```python
from build123d import *
from OCP.BRepFilletAPI import BRepFilletAPI_MakeChamfer

# Parameters (mm, degrees)
SKETCH1_R        = 10.376
BASENUT_DEPTH    = 38
ENDCHAMFER_SIZE  = 1.0376
ENDCHAMFER_SIZE2 = 0.599058639


with BuildPart() as part:
    # Sketch1 → BaseNut (new body)
    with BuildSketch(Plane.XY):
        Polygon((10.392304845, -18), (20.784609691, 0), (10.392304845, 18), (-10.392304845, 18), (-20.784609691, 0), (-10.392304845, -18), align=None)
        Circle(SKETCH1_R, mode=Mode.SUBTRACT)
    extrude(amount=-BASENUT_DEPTH)

    # Sketch2 → Double-Chamfer (revolve, cut)
    with BuildSketch(Plane(origin=(0, 0, 0), x_dir=(1, 0, 0), z_dir=(0, 1, 0))):
        Polygon((-20.784609691, 38), (-17.625, 38), (-20.784609691, 36.175798494), align=None)
        Polygon((-20.784609691, 1.824201506), (-20.784609691, 0), (-17.625, 0), align=None)
    revolve(axis=Axis((0, 0, -3.375940562), (0, 0, 1)), mode=Mode.SUBTRACT)

    # EndChamfer: one chamfer whose edges measure the first distance from different faces: ONE call of the kernel's chamfer builder (chamfer() names one face for all edges)
    endchamfer_edges_1 = [part.edges().sort_by_distance(p)[0] for p in [
        (-10.376, 0, -38),
    ]]
    endchamfer_side_1 = [part.faces().sort_by_distance(p)[0] for p in [
        (-10.376, 0, -19),
    ]]
    endchamfer_edges_2 = [part.edges().sort_by_distance(p)[0] for p in [
        (-10.376, 0, 0),
    ]]
    endchamfer_side_2 = [part.faces().sort_by_distance(p)[0] for p in [
        (17.126489719, 0, 0),
    ]]
    endchamfer = BRepFilletAPI_MakeChamfer(part.part.solid().wrapped)
    for e in endchamfer_edges_1:
        endchamfer.Add(ENDCHAMFER_SIZE, ENDCHAMFER_SIZE2, e.wrapped, endchamfer_side_1[0].wrapped)  # the first distance lies on this face
    for e in endchamfer_edges_2:
        endchamfer.Add(ENDCHAMFER_SIZE, ENDCHAMFER_SIZE2, e.wrapped, endchamfer_side_2[0].wrapped)  # the first distance lies on this face
    add(Compound.cast(endchamfer.Shape()), mode=Mode.REPLACE)


solid = part.part
```
CAD build for the part. Positions are in the model's coordinates, mm. Round coordinates to 2 decimals unless told otherwise and drop trailing zeros. Write each loop counter-clockwise with the first axis right and the second up, starting at its lowest first coordinate (ties: lowest second). Pieces come first, ordered by that corner, then holes. Notation, with made-up numbers: (73, -31.75) - (104, -31.75) arc R32 ccw to (104, 7.25) - close; hole circle Ø9 at (26.25, 18.25). An arc over 180 degrees is marked (long way). Return JSON: item names as keys, results as strings. Group by question number.
Item 1: Band-saw the part on B-B on z = -19.5. List the corners of the cut face in (x, y), plus the area to 3 significant figures.
Item 2: Flat gauge pins, fed straight in: pin 1 Ø5 at (y, z) = (-5, -23.5) entering from +X; pin 2 Ø2 at (x, y) = (-5.5, -8) entering from -Z; pin 3 Ø1.5 at (x, z) = (14, -18) entering from +Y. Where does each tip first touch, or does it go through?
Item 3: Mould opens along X. For faces 1 (the face through (-7.65, 7.01, -18.53)), 2 (the face through (3.864, 17.399, -0.114)), 3 (the face through (0, 18, -19)) say: +X half, -X half, draft (parallel to the pull), parting line (faces both ways), or undercut.
Item 4: Probe probe 1 along Y at (x, z) = (0, -8); probe 2 along Y at (x, z) = (7, -9.5); probe 3 along X at (y, z) = (-8.5, -18.5). List the from-to ranges inside material, lowest first.
Item 5: Band-saw the part on A-A on x = 0. List the corners of the cut face in (y, z) (1 decimal).
Resolved:
{
 "1": {"outline": "(-20.78, 0) - (-10.39, -18) - (10.39, -18) - (20.78, 0) - (10.39, 18) - (-10.39, 18) - close; hole circle Ø20.75 at (0, 0)", "area": "784 mm²"},
 "2": {"pin 1": "stops at x = 19.34", "pin 2": "stops at z = -37.54", "pin 3": "stops at y = 13.05"},
 "3": {"face 1": "undercut", "face 2": "parting line", "face 3": "draft"},
 "4": {"probe 1": "y = -18 to -10.38, 10.38 to 18", "probe 2": "y = -18 to -7.66, 7.66 to 18", "probe 3": "x = -15.88 to -5.95, 5.95 to 15.88"},
 "5": {"outline": "(-18, -37.8) - (-17.6, -38) - (-11, -38) - (-10.4, -37) - (-10.4, -0.6) - (-11.4, 0) - (-17.6, 0) - (-18, -0.2) - close; (10.4, -37) - (11, -38) - (17.6, -38) - (18, -37.8) - (18, -0.2) - (17.6, 0) - (11.4, 0) - (10.4, -0.6) - close"}
}
